For this review, take the finished solid that the model builds, in its own axes (mm). Coordinates: 2 decimals unless noted, no trailing zeros. Loops run counter-clockwise (first coordinate to the right, second up) from the corner with the lowest first, then second, coordinate; pieces in that order, holes last. Notation, with made-up numbers: M 2,67 L 20,67 A20 cw 20,100 Z; hole C 46,25 d2. An arc over 180 degrees is marked long. Answer as a JSON object with one key per item and string values. Group by question number.
Item 1: Wall thickness on L1, parallel to Y at x = -584.2, z = -0.2; L2, parallel to X at y = -146.5, z = 0.75; L3, parallel to Y at x = -1326.5, z = -0.1: over which ranges is each line inside the solid? List them lowest first. Write a range as from..to.
Item 2: Add section B-B (y = -12). State the section outline as (x, z) points, then the cut area to 3 significant figures.
Item 3: Add section A-A (z = -0.65). State the section outline as (x, y) points (3 decimals), then the cut area to 4 significant figures.
Item 4: Insertion check: pin 1 (0.6 mm diameter, centred on y = -131.5, z = 0, fed in from +X); pin 2 (0.6 mm diameter, centred on x = -1385.5, z = -0.5, fed in from -Y). Each pin has a flat end and moves straight along its axis. Give the tip position at first contact, or say it passes through.
Item 5: Add section D-D (y = 127.5). State the section outline as (x, z) points.
Item 6: Add section C-C (x = -1369.5). State the section outline as (y, z) points.
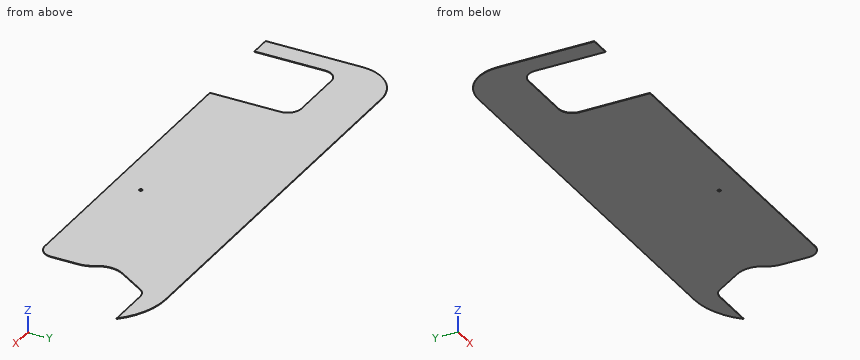
from build123d import *

# Parameters (mm, degrees)
SKETCH1_R           = 5.588
BOSS_EXTRUDE1_DEPTH = 1


with BuildPart() as part:
    # Sketch1 → Boss-Extrude1 (new, symmetric)
    with BuildSketch(Plane.XY):
        with BuildLine():
            Line((186.235876243, 172.72), (25.4, 172.72))
            ThreePointArc((25.4, 172.72), (1.035545712, 166.495928114), (-17.35858909, 149.348872727))
            Line((-17.35858909, 149.348872727), (-80.172354543, 51.429136363))
            ThreePointArc((-80.172354543, 51.429136363), (-95.248979697, 0.440870364), (-80.645, -50.684775574))
            ThreePointArc((-80.645, -50.684775574), (-69.764050811, -74.996020383), (-66.04, -101.369551148))
            Line((-66.04, -101.369551148), (-66.04, -203.2))
            ThreePointArc((-66.04, -203.2), (-80.918975516, -239.121024484), (-116.84, -254))
            Line((-116.84, -254), (-1244.6, -254))
            Line((-1244.6, -254), (-1244.6, 5.08))
            ThreePointArc((-1244.6, 5.08), (-1259.478975516, 41.001024484), (-1295.4, 55.88))
            Line((-1295.4, 55.88), (-1498.6, 55.88))
            ThreePointArc((-1498.6, 55.88), (-1534.521024484, 41.001024484), (-1549.4, 5.08))
            Line((-1549.4, 5.08), (-1549.4, -254))
            Line((-1549.4, -254), (-1625.6, -254))
            Line((-1625.6, -254), (-1625.6, 101.6))
            ThreePointArc((-1625.6, 101.6), (-1580.963073453, 209.363073453), (-1473.2, 254))
            Line((-1473.2, 254), (0, 254))
            ThreePointArc((0, 254), (101.6, 232.794845304), (186.235876243, 172.72))
        make_face()
        with Locations((-584.2, -152.4)):
            Circle(SKETCH1_R, mode=Mode.SUBTRACT)
    extrude(amount=BOSS_EXTRUDE1_DEPTH, both=True)


solid = part.part
From the geometry:
{
 "1": {"L1": "y = -254..-157.99, -146.81..254", "L2": "x = -1625.6..-1549.4, -1244.6..-66.04", "L3": "y = 55.88..254"},
 "2": {"outline": "M -1625.6,-1 L -1549.4,-1 L -1549.4,1 L -1625.6,1 Z; M -1244.6,-1 L -94.49,-1 L -94.49,1 L -1244.6,1 Z", "area": "2,450 mm²"},
 "3": {"outline": "M -1625.6,-254 L -1549.4,-254 L -1549.4,5.08 A50.8 cw -1498.6,55.88 L -1295.4,55.88 A50.8 cw -1244.6,5.08 L -1244.6,-254 L -116.84,-254 A50.8 ccw -66.04,-203.2 L -66.04,-101.37 A95.25 ccw -80.645,-50.685 A95.25 cw -80.172,51.429 L -17.359,149.349 A50.8 cw 25.4,172.72 L 186.236,172.72 A254 ccw 0,254 L -1473.2,254 A152.4 ccw -1625.6,101.6 Z; hole C -584.2,-152.4 d11.176", "area": "709,500 mm²"},
 "4": {"pin 1": "stops at x = -66.04", "pin 2": "stops at y = 55.88"},
 "5": {"outline": "M -1623.38,-1 L -31.37,-1 L -31.37,1 L -1623.38,1 Z"},
 "6": {"outline": "M 55.88,-1 L 254,-1 L 254,1 L 55.88,1 Z"}
}
